Geometry: see drawing. Coordinates: mm, zero at the bounding-box minimum. A direction names the side the tool comes from. Round coordinates to 2 decimals unless told otherwise and drop trailing zeros. Write each loop counter-clockwise with the first axis right and the second up, starting at its lowest first coordinate (ties: lowest second). Pieces come first, ordered by that corner, then holes. Notation, with made-up numbers: M 53.25,33.5 L 72.25,33.5 A29 ccw 72.25,63.5 Z; hole C -12,19 d10. An arc over 180 degrees is marked long. Use one line per item in the form item = value. Start each with the question number.
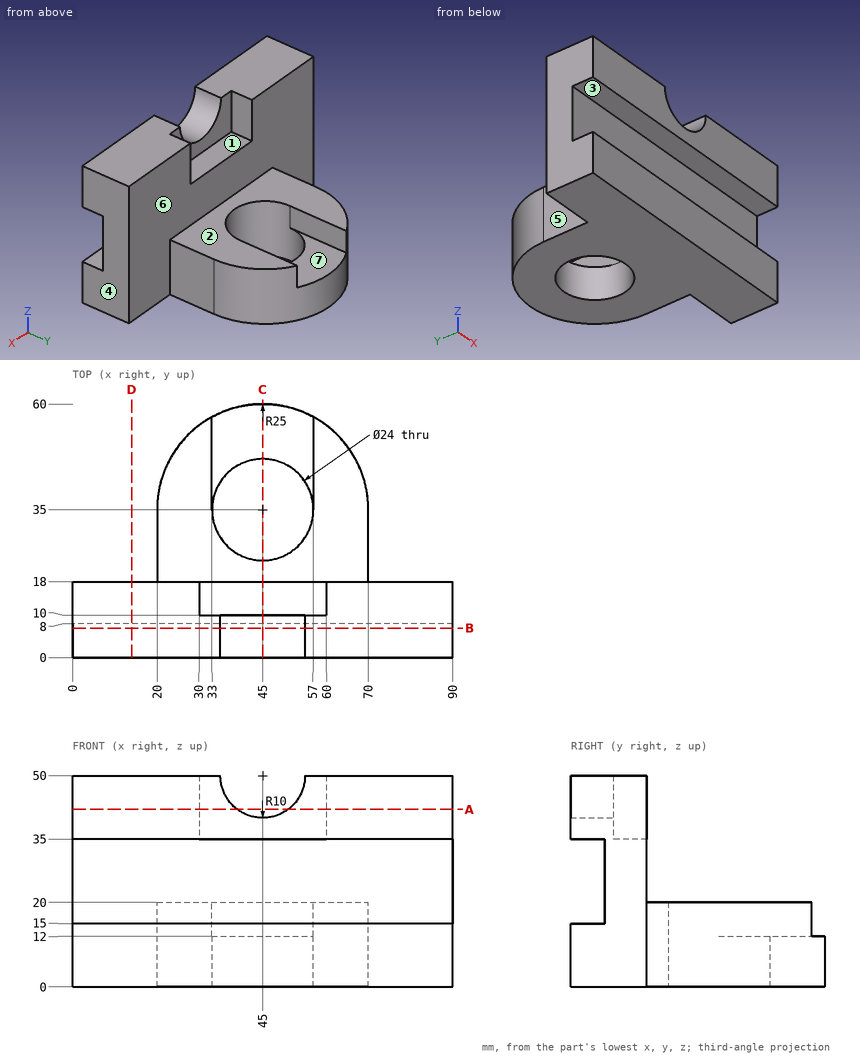
Item 1: Cut plane C-C (x = 45). Output: boundary loops of the cut face in (y, z), plus the area to 3 significant figures.
Item 2: Draft query along X for the marked faces 4, 5, 6 and 7. Return one class per face: +X half, -X half, draft (parallel to the pull), parting line (faces both ways), or undercut.
Item 3: First-contact query: pin 1 (6.5 mm diameter, centred on x = 35.5, y = 2.5, fed in from +Z); pin 2 (12 mm diameter, centred on x = 44, y = 44, fed in from +Z); pin 3 (8.5 mm diameter, centred on y = 26, z = 12.5, fed in from -X); pin 4 (4 mm diameter, centred on x = 48.5, y = 15.5, fed in from +Z). Flat tips, straight axial feed; report the tip coordinate or a pass-through.
Item 4: Cut plane B-B (y = 7). Output: boundary loops of the cut face in (x, z), plus the area to 3 significant figures.
Item 5: Reachability of the marked faces 1, 2 and 3 from +Z, -Z, +X, -X, +Y, -Y: full face, straight path, thin tool, end or side. Return the list, or none.
Item 6: Cut plane A-A (z = 42). Output: boundary loops of the cut face in (x, y), plus the area to 3 significant figures.
Item 7: Cut plane D-D (x = 14). Output: boundary loops of the cut face in (y, z).
Item 8: Ray query, line 1 (X direction, y = 35, z = 13); line 2 (X direction, y = 13, z = 39); line 3 (Y direction, x = 45, z = 6). Return the intervals inside material, ascending. Write a range as from..to.
Final values:
q1.outline = M 0,0 L 23,0 L 23,20 L 18,20 L 18,35 L 10,35 L 10,40 L 0,40 L 0,35 L 8,35 L 8,15 L 0,15 Z; M 47,0 L 60,0 L 60,12 L 47,12 Z
q1.area = 776 mm^2
q2.face_4 = +X half
q2.face_5 = -X half
q2.face_6 = draft
q2.face_7 = undercut
q3.pin_1 = 50
q3.pin_2 = 12
q3.pin_3 = 20
q3.pin_4 = 35
q4.outline = M 0,0 L 90,0 L 90,15 L 0,15 Z; M 0,35 L 90,35 L 90,50 L 55,50 A10 cw 35,50 L 0,50 Z
q4.area = 2,540 mm^2
q5.face_1 = +Z, +Y
q5.face_2 = +Z, +X, -X, +Y
q5.face_3 = +X, -X, -Y
q6.outline = M 0,0 L 39,0 L 39,10 L 30,10 L 30,18 L 0,18 Z; M 51,0 L 90,0 L 90,18 L 60,18 L 60,10 L 51,10 Z
q6.area = 1,260 mm^2
q7.outline = M 0,0 L 18,0 L 18,50 L 0,50 L 0,35 L 8,35 L 8,15 L 0,15 Z
q8.line_1 = 20..33, 57..70
q8.line_2 = 0..30, 60..90
q8.line_3 = 0..23, 47..60
